CAD build for the part. Positions are in the model's coordinates, mm. A direction names the side the tool comes from. Give positions to 0.01 mm unless a question says otherwise; leave off trailing zeros. Loops run counter-clockwise (first coordinate to the right, second up) from the corner with the lowest first, then second, coordinate; pieces in that order, holes last. Notation, with made-up numbers: M -34.5,2 L -19.5,2 A23 cw -19.5,28 Z; hole C 5.5,27.5 d4. An arc over 180 degrees is marked long. One line per question, with ' | ' between items.
```python
from build123d import *

# Parameters (mm, degrees)
BASE_PLATE_DEPTH            = 20
UPRIGHT_WALL_SKETCH_W       = 20
UPRIGHT_WALL_SKETCH_H       = 140
UPRIGHT_WALL_DEPTH          = 56
WALL_PROFILE_CUT_SKETCH_W   = 6
WALL_PROFILE_CUT_SKETCH_H   = 38
WALL_PROFILE_CUT_DEPTH      = 56
WALL_SLOT_DEPTH             = 56
TOP_RIDGE_SKETCH_W          = 36
TOP_RIDGE_SKETCH_H          = 46
TOP_RIDGE_DEPTH             = 36
WALL_NOTCH_SKETCH_W         = 30
WALL_NOTCH_SKETCH_H         = 10
WALL_NOTCH_DEPTH            = 22
ROUND_CUT_SKETCH_R          = 6
ROUND_CUT_DEPTH             = 65
STEP_CUT_SKETCH_W           = 10
STEP_CUT_SKETCH_H           = 20
STEP_CUT_DEPTH              = 65
STEP_CHAMFER_5MM_SIZE       = 5
BASE_EDGE_CHAMFER_5X45_SIZE = 5
CORNER_FILLET_R5_R          = 5
RIDGE_SLOT_DEPTH            = 65


with BuildPart() as part:
    # Base Plate Sketch → Base Plate (new body)
    with BuildSketch(Plane(origin=(0, 0, 0), x_dir=(1, 0, 0), z_dir=(0, 1, 0))):
        Polygon((28, 0), (28, 70), (-28, 70), (-28, -70), (28, -70), align=None)
    extrude(amount=BASE_PLATE_DEPTH)

    # Upright Wall Sketch → Upright Wall (add)
    with BuildSketch(Plane(origin=(0, 20, 0), x_dir=(1, 0, 0), z_dir=(0, 1, 0))):
        with Locations((18, 0)):
            Rectangle(UPRIGHT_WALL_SKETCH_W, UPRIGHT_WALL_SKETCH_H)
    extrude(amount=UPRIGHT_WALL_DEPTH)

    # Wall Profile Cut Sketch → Wall Profile Cut (cut)
    with BuildSketch(Plane(origin=(0, 76, 0), x_dir=(1, 0, 0), z_dir=(0, 1, 0))):
        with Locations((11, -51)):
            Rectangle(WALL_PROFILE_CUT_SKETCH_W, WALL_PROFILE_CUT_SKETCH_H)
    extrude(amount=-WALL_PROFILE_CUT_DEPTH, mode=Mode.SUBTRACT)

    # Wall Slot Sketch → Wall Slot (cut)
    with BuildSketch(Plane.ZY.offset(-14)):
        with BuildLine():
            Line((57, 64), (57, 34))
            ThreePointArc((57, 34), (51, 28), (45, 34))
            Line((45, 34), (45, 64))
            ThreePointArc((45, 64), (51, 70), (57, 64))
        make_face()
    extrude(amount=-WALL_SLOT_DEPTH, mode=Mode.SUBTRACT)

    # Top Ridge Sketch → Top Ridge (add)
    with BuildSketch(Plane.ZY.offset(28)):
        with Locations((-52, 23)):
            Rectangle(TOP_RIDGE_SKETCH_W, TOP_RIDGE_SKETCH_H)
    extrude(amount=-TOP_RIDGE_DEPTH)

    # Wall Notch Sketch → Wall Notch (cut)
    with BuildSketch(Plane.ZY.offset(28)):
        with Locations((-4, 15)):
            Rectangle(WALL_NOTCH_SKETCH_W, WALL_NOTCH_SKETCH_H)
    extrude(amount=-WALL_NOTCH_DEPTH, mode=Mode.SUBTRACT)

    # Round Cut Sketch → Round Cut (cut)
    with BuildSketch(Plane(origin=(0, 20, 0), x_dir=(1, 0, 0), z_dir=(0, 1, 0))):
        with Locations(Location((-17, 4, 0), (0, 0, 270))):
            Circle(ROUND_CUT_SKETCH_R)
    extrude(amount=-ROUND_CUT_DEPTH, mode=Mode.SUBTRACT)

    # Step Cut Sketch → Step Cut (cut)
    with BuildSketch(Plane.ZY.offset(-8)):
        with Locations((-65, 66)):
            Rectangle(STEP_CUT_SKETCH_W, STEP_CUT_SKETCH_H)
    extrude(amount=-STEP_CUT_DEPTH, mode=Mode.SUBTRACT)

    # Step Chamfer 5mm
    step_chamfer_5mm_edges = [part.edges().sort_by_distance(p)[0] for p in [
        (8, 66, -60),
    ]]
    chamfer(step_chamfer_5mm_edges, length=STEP_CHAMFER_5MM_SIZE)

    # Base Edge Chamfer 5x45
    base_edge_chamfer_5x45_edges = [part.edges().sort_by_distance(p)[0] for p in [
        (28, 66, -60),
    ]]
    chamfer(base_edge_chamfer_5x45_edges, length=BASE_EDGE_CHAMFER_5X45_SIZE)

    # Corner Fillet R5
    corner_fillet_r5_edges = [part.edges().sort_by_distance(p)[0] for p in [
        (28, 38, 70),
    ]]
    fillet(corner_fillet_r5_edges, radius=CORNER_FILLET_R5_R)

    # Ridge Slot Sketch → Ridge Slot (cut)
    with BuildSketch(Plane.XY.offset(-34)):
        with BuildLine():
            Line((-18.5, 39), (-1.5, 39))
            ThreePointArc((-1.5, 39), (4.5, 33), (-1.5, 27))
            Line((-1.5, 27), (-18.5, 27))
            ThreePointArc((-18.5, 27), (-24.5, 33), (-18.5, 39))
        make_face()
    extrude(amount=-RIDGE_SLOT_DEPTH, mode=Mode.SUBTRACT)


solid = part.part
```
Item 1: Saw through at B-B on x = -17. Give the cut face in (y, z), and give its area (3 significant figures).
Conclusion:
outline: M 0,-70 L 27,-70 L 27,-34 L 20,-34 L 20,-19 L 10,-19 L 10,-10 L 0,-10 Z; M 0,2 L 10,2 L 10,11 L 20,11 L 20,70 L 0,70 Z; M 39,-70 L 46,-70 L 46,-34 L 39,-34 Z | area: 2,880 mm²
Item 2: Saw through at C-C on y = 61. Give the cut face in (x, z), and give its area (3 significant figures).
Conclusion:
outline: M 8,-55 L 13,-60 L 23,-60 L 28,-55 L 28,45 L 14,45 L 14,32 L 8,32 Z; M 14,57 L 28,57 L 28,65 A5 ccw 23,70 L 14,70 Z | area: 2,170 mm²
Item 3: Mould opens along Z. For faces 6 (the flat face through (-28, 7, -17)), 7 (the flat face through (-17, 15, -19)), 8 (the flat face through (25, 66, -58)) say: pulls with the +Z half, pulls with the -Z half, needs draft (parallel to the pull), parting line crosses it, or undercut.
Conclusion:
face 6: needs draft | face 7: undercut | face 8: pulls with the -Z half
Item 4: Saw through at A-A on z = 51. Give the cut face in (x, y).
Conclusion:
outline: M -28,0 L 28,0 L 28,28 L 14,28 L 14,20 L -28,20 Z; M 14,70 L 28,70 L 28,76 L 14,76 Z
Item 5: Drill centre lines: line 1 along Z through (x, y) = (-18.5, 13); line 2 along X through (y, z) = (2.5, -4); line 3 along Y through (x, z) = (21, -61.5). Where is each one in solid material? Low to high. Write a range as [from, to].
Conclusion:
line 1: [-70, -19], [11, 70] | line 2: [-28, -23], [-11, 28] | line 3: [0, 56]
Item 6: Drop flat-ended pins along their axis: P1, Ø18, axis at x = -4, z = -54, coming from the +Y side; P2, Ø12, axis at x = 3, y = 60.5, coming from the -Z side; P3, Ø11.5, axis at y = 39.5, z = 47.5, coming from the -X side. Give the stop position or say it passes through.
Conclusion:
P1: y = 46 | P2: z = -56 | P3: x = 14
Item 7: Saw through at D-D on x = 2. Give the cut face in (y, z), and give its area (3 significant figures).
Conclusion:
outline: M 0,-70 L 28.13,-70 L 28.13,-34 L 20,-34 L 20,70 L 0,70 Z; M 37.87,-70 L 46,-70 L 46,-34 L 37.87,-34 Z | area: 3,390 mm²
Item 8: 3-axis set-ups, long thin cutter, end or side, ignore diameter. For faces 1 (the flat face through (11, 48, 32)), 2 (the flat face through (11, 66, -58)), 3 (the cylindrical face through (21, 70, 51)), 4 (the cylindrical face through (-24.5, 32.9, -51.7)), 5 (the flat face through (-17, 15, 11)): which of +Z, -Z, +X, -X, +Y, -Y reach the whole face in a straight line?
Conclusion:
face 1: +Z, -X, +Y | face 2: -Z, -X, +Y | face 3: +X, -X | face 4: +Z, -Z | face 5: -X, +Y
